Geometry: final body of the model. Coordinates: model frame, mm. Face numbers are marked on the shaded views. A direction names the side the tool comes from. Give positions to 0.01 mm unless a question says otherwise; leave off trailing zeros. Write each loop counter-clockwise with the first axis right and the second up, starting at its lowest first coordinate (ties: lowest second). Pieces come first, ordered by that corner, then holes. Notation, with made-up numbers: M 54.5,21 L 63.5,21 A21 cw 63.5,59 Z; hole C 49.25,-21.5 d6. An arc over 180 degrees is marked long. Answer as a JSON object with one key per item and string values.
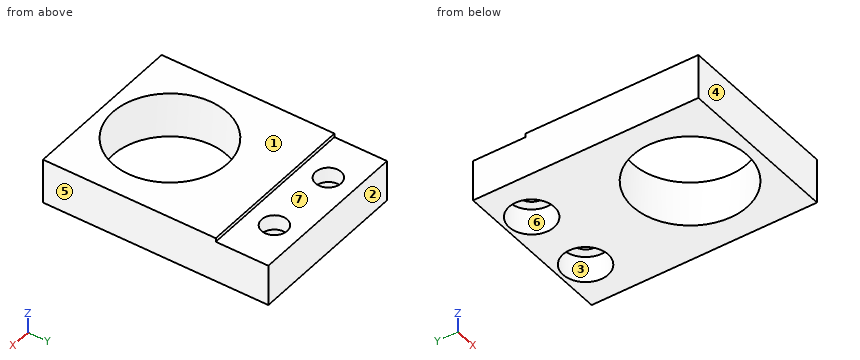
from build123d import *

# Parameters (mm, degrees)
SKETCH_1_W          = 22
SKETCH_1_H          = 30
SKETCH_1_R          = 7.615
SKETCH_1_R_2        = 1.7
EXTRUDE_1_DEPTH     = 6
SKETCH_3_W          = 0.5
SKETCH_3_H          = 7
CUT_EXTRUDE_1_DEPTH = 28.788445632
SKETCH_4_R          = 3
CUT_EXTRUDE_2_DEPTH = 3.5


with BuildPart() as part:
    # 草图1 → 凸台-拉伸1 (new body)
    with BuildSketch(Plane.XY):
        with Locations((-1.935779817, -0.880733945)):
            Rectangle(SKETCH_1_W, SKETCH_1_H)
        with Locations((-1.935779817, -6.880733945)):
            Circle(SKETCH_1_R, mode=Mode.SUBTRACT)
        with Locations((-6.935779817, 10.619266055)):
            Circle(SKETCH_1_R_2, mode=Mode.SUBTRACT)
        with Locations((3.064220183, 10.619266055)):
            Circle(SKETCH_1_R_2, mode=Mode.SUBTRACT)
    extrude(amount=EXTRUDE_1_DEPTH)

    # 草图3 → 切除-拉伸1 (cut, through all)
    with BuildSketch(Plane.ZY.offset(12.935779817)):
        with Locations((5.75, 10.619266055)):
            Rectangle(SKETCH_3_W, SKETCH_3_H)
    extrude(amount=-CUT_EXTRUDE_1_DEPTH, mode=Mode.SUBTRACT)

    # 草图4 → 切除-拉伸2 (cut)
    with BuildSketch(Plane(origin=(0, 0, 0), x_dir=(-1, 0, 0), z_dir=(0, 0, -1))):
        with Locations((-3.064220183, 10.619266055)):
            Circle(SKETCH_4_R)
        with Locations((6.935779817, 10.619266055)):
            Circle(SKETCH_4_R)
    extrude(amount=-CUT_EXTRUDE_2_DEPTH, mode=Mode.SUBTRACT)


solid = part.part
1) Cut plane A-A on y = -14. Return loops of the section in (x, z), and give its area (3 significant figures).
Geometry check:
{"outline": "M -12.94,0 L -4.64,0 L -4.64,6 L -12.94,6 Z; M 0.77,0 L 9.06,0 L 9.06,6 L 0.77,6 Z", "area": "99.6 mm2"}
2) Line query: line 1 (Y direction, x = -6, z = 1.3); line 2 (X direction, y = 12.25, z = 2.65); line 3 (Y direction, x = -7.5, z = 0.7). Output: solid intervals per line, ascending. Write a range as from..to.
Geometry check:
{"line 1": "y = -15.88..-13.32, -0.44..7.77, 13.47..14.12", "line 2": "x = -12.94..-9.45, -4.42..0.55, 5.58..9.06", "line 3": "y = -15.88..-12.08, -1.68..7.67, 13.57..14.12"}
3) Cut plane D-D on y = 11. Return loops of the section in (x, z), and give its area (3 significant figures).
Geometry check:
{"outline": "M -12.94,0 L -9.91,0 L -9.91,3.5 L -8.59,3.5 L -8.59,5.5 L -12.94,5.5 Z; M -5.28,3.5 L -3.96,3.5 L -3.96,0 L 0.09,0 L 0.09,3.5 L 1.41,3.5 L 1.41,5.5 L -5.28,5.5 Z; M 4.72,3.5 L 6.04,3.5 L 6.04,0 L 9.06,0 L 9.06,5.5 L 4.72,5.5 Z", "area": "66.1 mm2"}
4) Contact query for flat-ended pins moving along their axis: P1, Ø5.5, axis at x = 3.06, y = 10.62, coming from the -Z side; P2, Ø4, axis at x = -6.94, y = 10.62, coming from the +Z side. Output: stop coordinate, or through.
Geometry check:
{"P1": "stops at z = 3.5", "P2": "stops at z = 5.5"}
5) Cut plane B-B on x = -3. Return loops of the section in (y, z), and give its area (3 significant figures).
Geometry check:
{"outline": "M -15.88,0 L -14.42,0 L -14.42,6 L -15.88,6 Z; M 0.66,0 L 14.12,0 L 14.12,5.5 L 7.12,5.5 L 7.12,6 L 0.66,6 Z", "area": "86.0 mm2"}
6) Cut plane C-C on z = 5.1. Return loops of the section in (x, y) (3 decimals), and give its area (3 significant figures).
Geometry check:
{"outline": "M -12.936,-15.881 L 9.064,-15.881 L 9.064,14.119 L -12.936,14.119 Z; hole C -1.936,-6.881 d15.23; hole C -6.936,10.619 d3.4; hole C 3.064,10.619 d3.4", "area": "460 mm2"}
7) Set-up query: the marked faces 5, 6 and 7. Return all of +Z, -Z, +X, -X, +Y, -Y with unobstructed straight access to the full face (end or side cutting, diameter ignored); none if empty.
Geometry check:
{"face 5": "+Z, -Z, +X, +Y, -Y", "face 6": "-Z", "face 7": "+Z, +X, -X, +Y"}
8) Pull-direction query (Y, two-part tool) for the marked faces 1, 2, 3 and 4; classes: pulls with the +Y half, pulls with the -Y half, needs draft (parallel to the pull), parting line crosses it, or undercut.
Geometry check:
{"face 1": "needs draft", "face 2": "pulls with the +Y half", "face 3": "undercut", "face 4": "pulls with the -Y half"}
